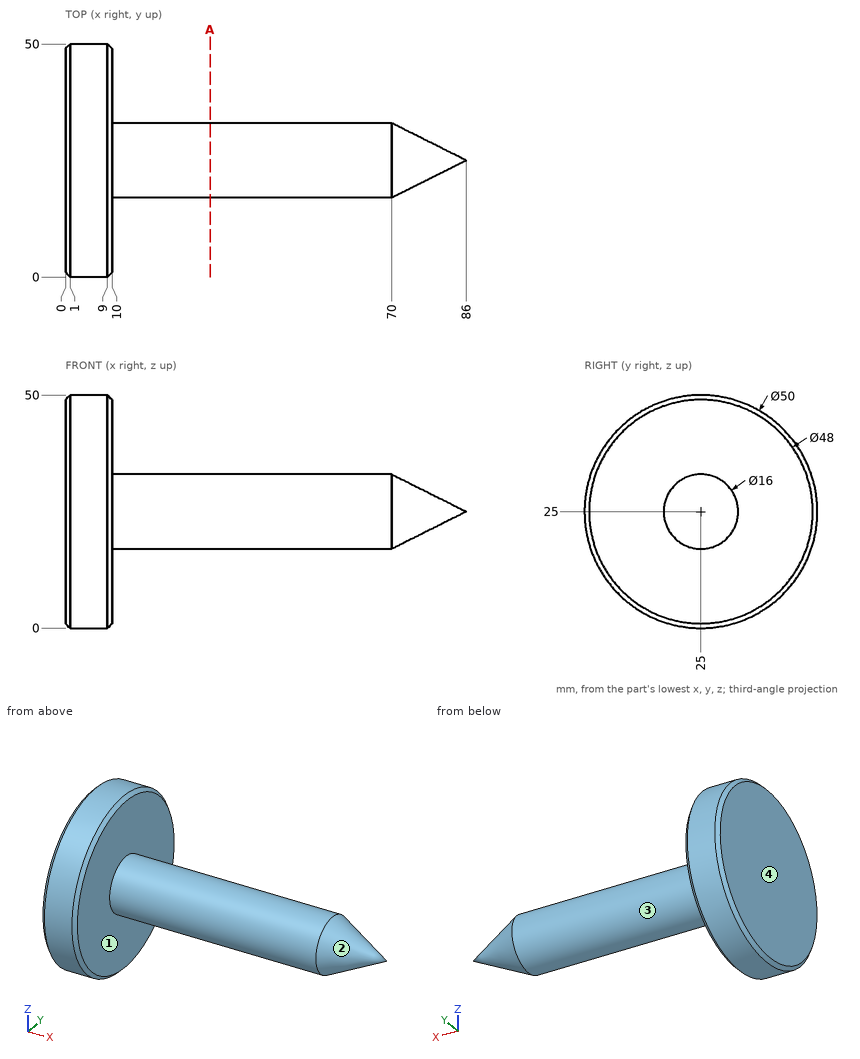
Geometry: see drawing. Coordinates: mm, zero at the bounding-box minimum. A direction names the side the tool comes from. Coordinates: 2 decimals unless noted, no trailing zeros. Loops run counter-clockwise (first coordinate to the right, second up) from the corner with the lowest first, then second, coordinate; pieces in that order, holes last.
(1) Section A-A on x = 31. Return the cut outline in (y, z).
(2) Material intervals for probe 1 along Z at (x, y) = (57, 25.5); probe 2 along X at (y, z) = (14.5, 24); probe 3 along Y at (x, z) = (28, 25), sorted ascending.
(3) Set-up query: the marked faces 3 and 4. Return all of +Z, -Z, +X, -X, +Y, -Y with unobstructed straight access to the full face (end or side cutting, diameter ignored); none if empty.
(4) First-contact query: pin 1 Ø3 at (y, z) = (22.5, 7) entering from -X; pin 2 Ø3 at (x, z) = (50, 19.5) entering from -Y; pin 3 Ø2 at (x, y) = (17, 22) entering from +Z; pin 4 Ø8 at (y, z) = (17.5, 9) entering from +X. Flat tips, straight axial feed; report the tip coordinate or a pass-through.
(5) Pull-direction query (Z, two-part tool) for the marked faces 1 and 2; classes: released by +Z, released by -Z, zero draft, split by the parting line, or undercut.
Data:
1. outline: circle Ø16 at (25, 25)
2. probe 1: z = 17.02 to 32.98
2. probe 2: x = 0 to 10
2. probe 3: y = 17 to 33
3. face 3: +X
3. face 4: +Z, -Z, -X, +Y, -Y
4. pin 1: stops at x = 0
4. pin 2: stops at y = 18.07
4. pin 3: stops at z = 32.75
4. pin 4: stops at x = 10
5. face 1: zero draft
5. face 2: split by the parting line
